Source: three-view drawing plus pictorial views. Frame: mm from the lowest corner of the part. A direction names the side the tool comes from. Coordinates: 2 decimals unless noted, no trailing zeros. Write each loop counter-clockwise with the first axis right and the second up, starting at its lowest first coordinate (ties: lowest second). Pieces come first, ordered by that corner, then holes. Notation, with made-up numbers: (18.5, -20.5) - (69.5, -20.5) arc R20 cw to (69.5, -5.5) - close; hole circle Ø7 at (58, 12.25). An arc over 180 degrees is marked (long way). Answer as a JSON object with one key per item and string values. Group by question number.
Item 1: Set-up query: the marked faces 4, 5 and 6. Return all of +Z, -Z, +X, -X, +Y, -Y with unobstructed straight access to the full face (end or side cutting, diameter ignored); none if empty.
Item 2: Line query: line 1 along Y through (x, z) = (5.75, 4.5); line 2 along Y through (x, z) = (2.25, 2.75); line 3 along X through (y, z) = (7, 2.25). Output: solid intervals per line, ascending. Write a range as from..to.
Item 3: Section A-A on y = 14.75. Return loops of the section in (x, z), and give its area (3 significant figures).
Item 4: First-contact query: pin 1 Ø3 at (x, y) = (3, 16) entering from -Z; pin 2 Ø4 at (y, z) = (12.5, 5.5) entering from +X; pin 3 Ø1.5 at (x, z) = (3, 3) entering from +Y; pin 4 Ø3.5 at (x, z) = (4.5, 5) entering from -Y. Flat tips, straight axial feed; report the tip coordinate or a pass-through.
Item 5: Mould query, pull axis X, two halves, no side actions, for the marked faces 1, 2 and 3. Classes: pulls with the +X half, pulls with the -X half, needs draft (parallel to the pull), parting line crosses it, or undercut.
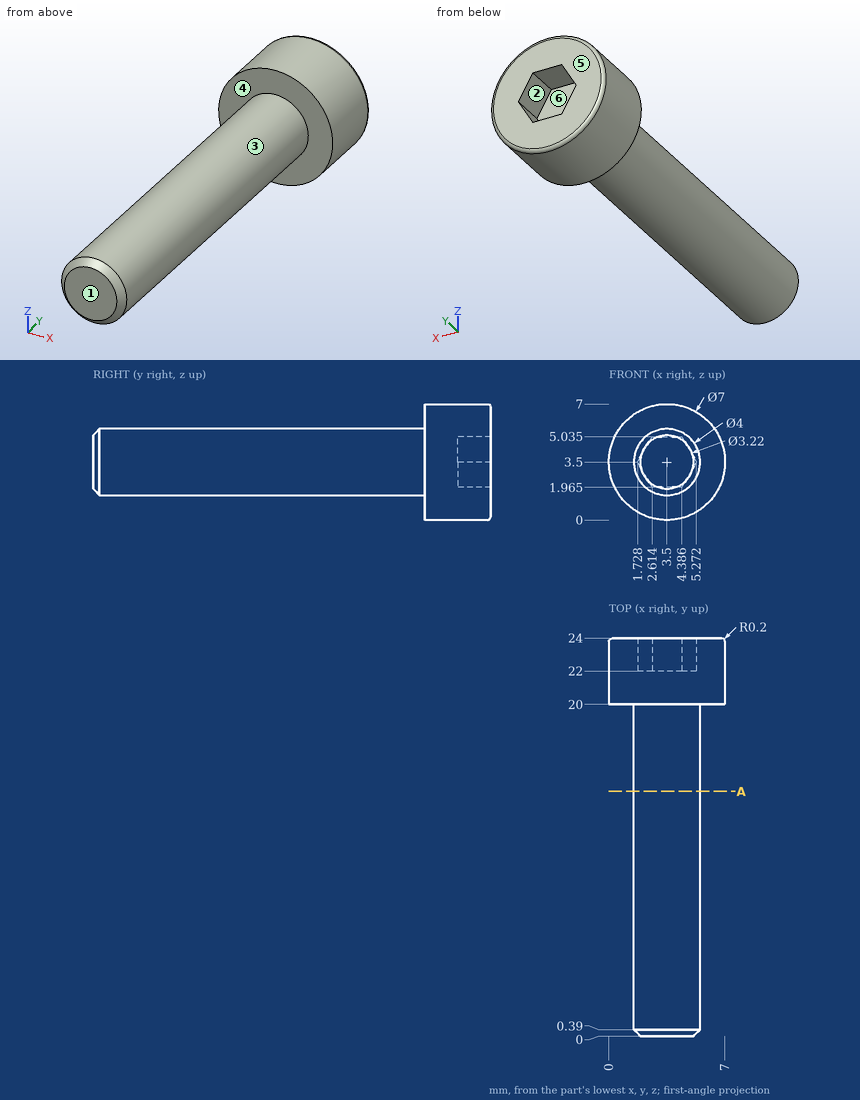
Checks:
{
 "1": {"face 4": "-Y", "face 5": "+Z, -Z, +X, -X, +Y", "face 6": "+Y"},
 "2": {"line 1": "20..24", "line 2": "0..22", "line 3": "1.94..5.06"},
 "3": {"outline": "circle Ø4 at (3.5, 3.5)", "area": "12.6 mm^2"},
 "4": {"pin 1": "z = 1.5", "pin 2": "x = 5.5", "pin 3": "y = 22", "pin 4": "y = 0"},
 "5": {"face 1": "needs draft", "face 2": "undercut", "face 3": "parting line crosses it"}
}
